from build123d import *

# Parameters (mm, degrees)
FLANGE_PROFILE_SKETCH_R   = 50
FLANGE_PROFILE_SKETCH_R_2 = 5.5
FLANGE_100_DEPTH          = 7.5
HUB_50_DEPTH              = 17.5
HUB_SLOTS_SKETCH_R        = 8.5
HUB_SLOTS_4X_DEPTH        = 7


with BuildPart() as part:
    # Flange Profile Sketch → Flange Ø100 (new, symmetric)
    with BuildSketch(Plane.XY):
        Circle(FLANGE_PROFILE_SKETCH_R)
        with Locations((-35, 0)):
            Circle(FLANGE_PROFILE_SKETCH_R_2, mode=Mode.SUBTRACT)
        with Locations((35, 0)):
            Circle(FLANGE_PROFILE_SKETCH_R_2, mode=Mode.SUBTRACT)
        with Locations((0, -35)):
            Circle(FLANGE_PROFILE_SKETCH_R_2, mode=Mode.SUBTRACT)
        with BuildLine():
            Line((-11.763017547, 12.956906196), (-11.763017547, 21))
            ThreePointArc((-11.763017547, 21), (-10.591444672, 23.828427125), (-7.763017547, 25))
            Line((-7.763017547, 25), (-5, 25))
            Line((-5, 25), (-5, 35))
            ThreePointArc((-5, 35), (0, 40), (5, 35))
            Line((5, 35), (5, 25))
            Line((5, 25), (9.236982453, 25))
            ThreePointArc((9.236982453, 25), (12.065409578, 23.828427125), (13.236982453, 21))
            Line((13.236982453, 21), (13.236982453, 11.446933893))
            ThreePointArc((13.236982453, 11.446933893), (-1.055057925, -17.468166841), (-11.763017547, 12.956906196))
        make_face(mode=Mode.SUBTRACT)
    extrude(amount=FLANGE_100_DEPTH, both=True)

    # Hub Profile Sketch → Hub Ø50 (add, symmetric)
    with BuildSketch(Plane.XY.offset(7.5)):
        with BuildLine():
            Line((-11.763017547, 12.956906196), (-11.763017547, 22.059723892))
            ThreePointArc((-11.763017547, 22.059723892), (-0.851158679, -24.985506377), (13.236982453, 21.208071472))
            Line((13.236982453, 21.208071472), (13.236982453, 11.446933893))
            ThreePointArc((13.236982453, 11.446933893), (-1.055057925, -17.468166841), (-11.763017547, 12.956906196))
        make_face()
    extrude(amount=HUB_50_DEPTH, both=True)

    # Hub Slots Sketch → Hub Slots 4x (cut)
    with BuildSketch(Plane.XY.offset(7.5)):
        with Locations((-35, 0)):
            Circle(HUB_SLOTS_SKETCH_R)
        with Locations((35, 0)):
            Circle(HUB_SLOTS_SKETCH_R)
        with Locations((0, -35)):
            Circle(HUB_SLOTS_SKETCH_R)
    extrude(amount=-HUB_SLOTS_4X_DEPTH, mode=Mode.SUBTRACT)


solid = part.part
Could you check a few things on this model? Use its own coordinates, in mm. A direction names the side the tool comes from. Round coordinates to 2 decimals unless told otherwise and drop trailing zeros. Write each loop counter-clockwise with the first axis right and the second up, starting at its lowest first coordinate (ties: lowest second). Pieces come first, ordered by that corner, then holes. Notation, with made-up numbers: (73, 49.25) - (100, 49.25) arc R10 cw to (100, 68.25) - close; hole circle Ø4 at (29, 14.5). An arc over 180 degrees is marked (long way). Put each result on its own line as item: value. Start each with the question number.
(1) I need wall thicknesses on probe 1 along Y at (x, z) = (0, 2); probe 2 along Z at (x, y) = (-43, -10); probe 3 along Y at (x, z) = (7, 6). Which ranges of each line are inside material? Lowest first, please.
(2) Will these pins go through, and if not, where does the flat tip stop? pin 1 (12 mm diameter, centred on y = 18.5, z = 19, fed in from +X); pin 2 (10 mm diameter, centred on x = 0, y = -35, fed in from +Z); pin 3 (7.5 mm diameter, centred on y = 17, z = 7.5, fed in from +X); pin 4 (15.5 mm diameter, centred on x = -35, y = 0, fed in from -Z).
(3) I want a section at B-B, the plane z = -6. Please give me the cut outline in (x, y).
(4) For faces 4 (the cylindrical face through (-1.84, -43.3, 4.05)), 5 (the cylindrical face through (12.034, 23.859, 0.105)), which set-ups out of +Z, -Z, +X, -X, +Y, -Y let a thin tool reach every point of the face, with its end or its side?
(5) I want a section at C-C, the plane y = 0. Give the number of separate pieces and of enclosed holes in the cut face, plus the area to 3 significant figures.
(6) I want a section at A-A, the plane x = 0. Please give me the cut outline in (y, z), plus the area to 4 significant figures.
(7) Thinking about a two-plate mould opening in X: for faces 1 (the cylindrical face through (-1.766, -24.938, -8.733)), 2 (the flat face through (-9.4, -15.3, -10)), 3 (the cylindrical face through (0, 40, 0)), which applies, released by +X, released by -X, zero draft, split by the parting line, or undercut?
(8) I want a section at D-D, the plane y = -35. Please give me the cut outline in (x, z), plus the area to 3 significant figures.
Here are the results:
1. probe 1: y = -50 to -43.5, -26.5 to -17.5, 40 to 50
1. probe 2: z = -7.5 to 7.5
1. probe 3: y = -49.51 to -39.82, -30.18 to -16.04, 25 to 49.51
2. pin 1: stops at x = 21.65
2. pin 2: passes through
2. pin 3: stops at x = 48.21
2. pin 4: stops at z = -7.5
3. outline: circle Ø100 at (0, 0); hole circle Ø11 at (-35, 0); hole (-11.76, 12.96) arc R17.5 ccw (long way) to (13.24, 11.45) - (13.24, 21) arc R4 ccw to (9.24, 25) - (5, 25) - (5, 35) arc R5 ccw to (-5, 35) - (-5, 25) - (-7.76, 25) arc R4 ccw to (-11.76, 21) - close; hole circle Ø11 at (0, -35); hole circle Ø11 at (35, 0)
4. face 4: +Z
4. face 5: +Z, -Z
5. separate pieces: 4
5. enclosed holes: 0
5. area: 861 mm^2
6. outline: (-50, -7.5) - (-40.5, -7.5) - (-40.5, 0.5) - (-43.5, 0.5) - (-43.5, 7.5) - (-50, 7.5) - close; (-29.5, -7.5) - (-25, -7.5) - (-25, -10) - (-17.5, -10) - (-17.5, 25) - (-25, 25) - (-25, 7.5) - (-26.5, 7.5) - (-26.5, 0.5) - (-29.5, 0.5) - close; (40, -7.5) - (50, -7.5) - (50, 7.5) - (40, 7.5) - close
6. area: 580.5 mm^2
7. face 1: split by the parting line
7. face 2: zero draft
7. face 3: undercut
8. outline: (-35.71, -7.5) - (-5.5, -7.5) - (-5.5, 0.5) - (-8.5, 0.5) - (-8.5, 7.5) - (-35.71, 7.5) - close; (5.5, -7.5) - (35.71, -7.5) - (35.71, 7.5) - (8.5, 7.5) - (8.5, 0.5) - (5.5, 0.5) - close
8. area: 864 mm^2
